```python
from build123d import *

# Parameters (mm, degrees)
SKETCH_1_R             = 12.5
EXTRUDE_1_DEPTH        = 590
HOLE_WIZARD_M8_1_D     = 6.8
HOLE_WIZARD_M8_1_DEPTH = 19.75
HOLE_WIZARD_M8_1_TIP   = 2.042926105
HOLE_WIZARD_M8_2_D     = 6.8
HOLE_WIZARD_M8_2_DEPTH = 19.75
HOLE_WIZARD_M8_2_TIP   = 2.042926105
CHAMFER_1_SIZE         = 0.5


with BuildPart() as part:
    # 草图1 → 凸台-拉伸1 (new body)
    with BuildSketch(Plane.XY):
        Circle(SKETCH_1_R)
    extrude(amount=EXTRUDE_1_DEPTH)

    # M8 螺纹孔1
    with Locations(Plane.XY.offset(590)):
        with Locations((0, 0)):
            Hole(HOLE_WIZARD_M8_1_D / 2, depth=HOLE_WIZARD_M8_1_DEPTH)
            with Locations((0, 0, -(HOLE_WIZARD_M8_1_DEPTH + HOLE_WIZARD_M8_1_TIP / 2))):  # 118° drill point
                Cone(0, HOLE_WIZARD_M8_1_D / 2, HOLE_WIZARD_M8_1_TIP, mode=Mode.SUBTRACT)

    # M8 螺纹孔2
    with Locations(Plane(origin=(0, 0, 0), x_dir=(-1, 0, 0), z_dir=(0, 0, -1))):
        with Locations((0, 0)):
            Hole(HOLE_WIZARD_M8_2_D / 2, depth=HOLE_WIZARD_M8_2_DEPTH)
            with Locations((0, 0, -(HOLE_WIZARD_M8_2_DEPTH + HOLE_WIZARD_M8_2_TIP / 2))):  # 118° drill point
                Cone(0, HOLE_WIZARD_M8_2_D / 2, HOLE_WIZARD_M8_2_TIP, mode=Mode.SUBTRACT)

    # 倒角1
    chamfer_1_edges = [part.edges().sort_by_distance(p)[0] for p in [
        (-3.4, 0, 0),
        (-12.5, 0, 0),
        (-12.5, 0, 590),
    ]]
    chamfer(chamfer_1_edges, length=CHAMFER_1_SIZE)


solid = part.part
```
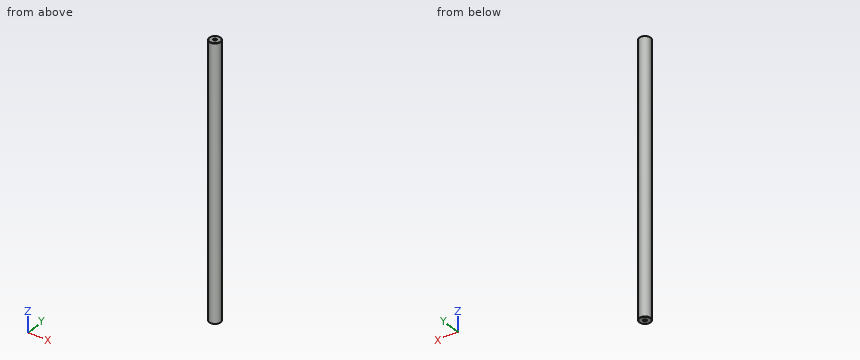
Geometry: final body of the model. Coordinates: model frame, mm. Coordinates: 2 decimals unless noted, no trailing zeros. Loops run counter-clockwise (first coordinate to the right, second up) from the corner with the lowest first, then second, coordinate; pieces in that order, holes last. Notation, with made-up numbers: (-1.75, -8) -> (12.25, -8) arc R14 ccw to (12.25, 6) -> close; hole circle Ø4 at (81, 89.5). An arc over 180 degrees is marked (long way). Use a Markdown table: item, result. Add a question column.
(1) Line query: line 1 along Y through (x, z) = (0, 4.5); line 2 along Y through (x, z) = (1.5, 409); line 3 along X through (y, z) = (1, 244). Output: solid intervals per line, ascending.
(2) Section query A-A, the plane z = 52.5. Return loops of the section in (x, y).
(3) Pin query (flat end, axial travel): pin 1 Ø2 at (y, z) = (7, 393) entering from -X; pin 2 Ø1.5 at (y, z) = (4.5, 488.5) entering from +X; pin 3 Ø4 at (x, y) = (0, 0) entering from +Z. Return the tip coordinate at first contact, or that it passes through.
Answer:
| question | item | result |
|---|---|---|
| 1 | line 1 | y = -12.5 to -3.4, 3.4 to 12.5 |
| 1 | line 2 | y = -12.41 to 12.41 |
| 1 | line 3 | x = -12.46 to 12.46 |
| 2 | outline | circle Ø25 at (0, 0) |
| 3 | pin 1 | stops at x = -10.97 |
| 3 | pin 2 | stops at x = 11.92 |
| 3 | pin 3 | stops at z = 569.41 |
